Design review of the part built by this model. Coordinates are the model's own, in mm. Face numbers are marked on the shaded views. A direction names the side the tool comes from. Coordinates: 2 decimals unless noted, no trailing zeros. Loops run counter-clockwise (first coordinate to the right, second up) from the corner with the lowest first, then second, coordinate; pieces in that order, holes last. Notation, with made-up numbers: (-17, -22.75) -> (-13, -22.75) arc R18 ccw to (-13, -1.75) -> close; hole circle Ø11 at (55.5, 44). An arc over 180 degrees is marked (long way). Use one line per item in the form item = value. Start each with the question number.
1. Consider section D-D (y = 22.75). State the section outline as (x, z) points (3 decimals).
2. For pin 1 (5.5 mm diameter, centred on y = 18.5, z = 6.5, fed in from -X); pin 2 (1 mm diameter, centred on y = 11.5, z = 15, fed in from +X); pin 3 (5 mm diameter, centred on y = 11, z = 5.5, fed in from +X), all flat-tipped, find the tip position at first contact; note any pin that passes through.
3. Machinability: for the marked faces 1, 2 and 3, which of the approach directions +Z, -Z, +X, -X, +Y, -Y give a long, thin tool a straight path to every point of the face, cutting with its end or side? Answer none if there is none.
4. Wall thickness on line 1 (X direction, y = 2.8, z = 12.5); line 2 (X direction, y = 18.25, z = 17); line 3 (Y direction, x = 16.5, z = 5): over which ranges is each line inside the solid? List them lowest first. Write a range as from..to.
5. The part is to be moulded in two halves that separate along X. For the marked faces 4, 5, 6 and 7, say which applies: released by +X, released by -X, zero draft, split by the parting line, or undercut.
6. Consider section A-A (z = 3). State the section outline as (x, y) points, then the cut area to 3 significant figures.
7. Consider section C-C (z = 14.25). State the section outline as (x, y) points, then the cut area to 3 significant figures.
8. Consider section B-B (x = 7.5). State the section outline as (y, z) points, then the cut area to 3 significant figures.
from build123d import *

# Parameters (mm, degrees)
BASE_PROFILE_SKETCH_W      = 40
BASE_PROFILE_SKETCH_H      = 6
BASE_BODY_DEPTH            = 25
UPRIGHT_BLOCK_SKETCH_W     = 6
UPRIGHT_BLOCK_SKETCH_H     = 15
UPRIGHT_BLOCK_DEPTH        = 25
SLOTTED_CLEVIS_PLATE_DEPTH = 6
LUG_1_DEPTH                = 5
LUG_1_PIN_HOLE_SKETCH_R    = 1.25
LUG_1_PIN_HOLE_DEPTH       = 5
LUG_START                  = -5
LUG_2_DEPTH                = 5
LUG_2_PIN_HOLE_SKETCH_R    = 1.25
LUG_2_PIN_HOLE_DEPTH       = 5
MOUNTING_HOLES_SKETCH_R    = 3
MOUNTING_HOLES_2X_6_DEPTH  = 6


with BuildPart() as part:
    # Base Profile Sketch → Base Body (new body)
    with BuildSketch(Plane.XY):
        with Locations((20, 3)):
            Rectangle(BASE_PROFILE_SKETCH_W, BASE_PROFILE_SKETCH_H)
    extrude(amount=BASE_BODY_DEPTH)

    # Upright Block Sketch → Upright Block (add)
    with BuildSketch(Plane.XY.offset(25)):
        with Locations((43, 7.5)):
            Rectangle(UPRIGHT_BLOCK_SKETCH_W, UPRIGHT_BLOCK_SKETCH_H)
    extrude(amount=-UPRIGHT_BLOCK_DEPTH)

    # Clevis Slot Profile Sketch → Slotted Clevis Plate (add)
    with BuildSketch(Plane.ZY.offset(-40)):
        with BuildLine():
            ThreePointArc((16, 18.5), (14.974873734, 16.025126266), (12.5, 15))
            Line((12.5, 15), (25, 15))
            Line((25, 15), (20, 25))
            Line((20, 25), (16, 25))
            Line((16, 25), (16, 18.5))
        make_face()
        with BuildLine():
            ThreePointArc((12.5, 15), (10.025126266, 16.025126266), (9, 18.5))
            Line((9, 18.5), (9, 25))
            Line((9, 25), (5, 25))
            Line((5, 25), (0, 15))
            Line((0, 15), (12.5, 15))
        make_face()
    extrude(amount=-SLOTTED_CLEVIS_PLATE_DEPTH)

    # Lug 1 Sketch → Lug 1 (add)
    with BuildSketch(Plane.XY.offset(25)):
        with BuildLine():
            Line((46, 0), (53, 0))
            ThreePointArc((53, 0), (55.757828687, 1.81916092), (55.171034593, 5.070412712))
            Line((55.171034593, 5.070412712), (46, 15))
            Line((46, 15), (46, 0))
        make_face()
    extrude(amount=-LUG_1_DEPTH)

    # Lug 1 Pin Hole Sketch → Lug 1 Pin Hole (cut)
    with BuildSketch(Plane.XY.offset(25)):
        with Locations((53, 3)):
            Circle(LUG_1_PIN_HOLE_SKETCH_R)
    extrude(amount=-LUG_1_PIN_HOLE_DEPTH, mode=Mode.SUBTRACT)

    # Lug 2 Sketch → Lug 2 (add)
    with BuildSketch(Plane(origin=(0, 0, 0), x_dir=(-1, 0, 0), z_dir=(0, 0, -1)).offset(LUG_START)):
        with BuildLine():
            Line((-46, 0), (-53, 0))
            ThreePointArc((-53, 0), (-55.757828687, 1.81916092), (-55.171034593, 5.070412712))
            Line((-55.171034593, 5.070412712), (-46, 15))
            Line((-46, 15), (-46, 0))
        make_face()
    extrude(amount=LUG_2_DEPTH)

    # Lug 2 Pin Hole Sketch → Lug 2 Pin Hole (cut)
    with BuildSketch(Plane(origin=(0, 0, 0), x_dir=(-1, 0, 0), z_dir=(0, 0, -1)).offset(LUG_START)):
        with Locations(Location((-53, 3, 0), (0, 0, 180))):
            Circle(LUG_2_PIN_HOLE_SKETCH_R)
    extrude(amount=LUG_2_PIN_HOLE_DEPTH, mode=Mode.SUBTRACT)

    # Mounting Holes Sketch → Mounting Holes 2xØ6 (cut)
    with BuildSketch(Plane(origin=(0, 6, 0), x_dir=(1, 0, 0), z_dir=(0, 1, 0))):
        with Locations(Location((7.5, -12.5, 0), (0, 0, 270))):
            Circle(MOUNTING_HOLES_SKETCH_R)
        with Locations(Location((25, -12.5, 0), (0, 0, 270))):
            Circle(MOUNTING_HOLES_SKETCH_R)
    extrude(amount=-MOUNTING_HOLES_2X_6_DEPTH, mode=Mode.SUBTRACT)


solid = part.part
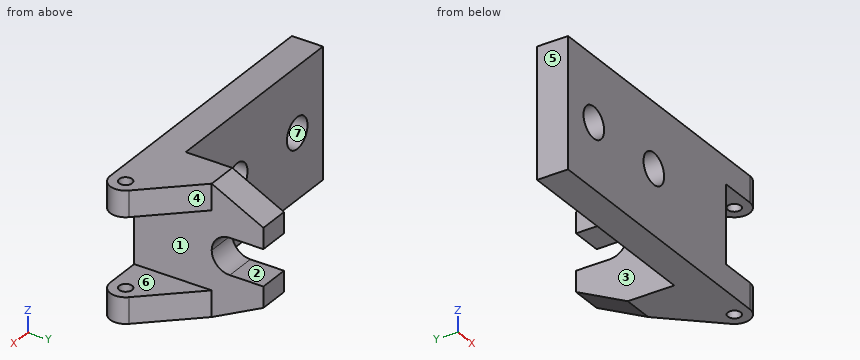
Geometry check:
q1.outline = (40, 3.875) -> (46, 3.875) -> (46, 9) -> (40, 9) -> close; (40, 16) -> (46, 16) -> (46, 21.125) -> (40, 21.125) -> close
q2.pin_1 = 40
q2.pin_2 = 46
q2.pin_3 = 51.96
q3.face_1 = +X, +Y
q3.face_2 = +X, -X, +Y
q3.face_3 = +Z, -Z, -X, +Y
q4.line_1 = 0..4.5, 10.5..22, 28..46
q4.line_2 = 40..46
q4.line_3 = 0..6
q5.face_4 = released by +X
q5.face_5 = released by -X
q5.face_6 = zero draft
q5.face_7 = undercut
q6.outline = (0, 0) -> (53, 0) arc R3 ccw to (55.17, 5.07) -> (46, 15) -> (46, 21) -> (40, 21) -> (40, 6) -> (0, 6) -> close; hole circle Ø2.5 at (53, 3)
q6.area = 455 mm²
q7.outline = (0, 0) -> (5.06, 0) -> (5.06, 6) -> (0, 6) -> close; (9.94, 0) -> (22.56, 0) -> (22.56, 6) -> (9.94, 6) -> close; (27.44, 0) -> (46, 0) -> (46, 15.47) -> (40, 15.47) -> (40, 6) -> (27.44, 6) -> close
q7.area = 274 mm²
q8.outline = (0, 0) -> (6, 0) -> (6, 9.5) -> (0, 9.5) -> close; (0, 15.5) -> (6, 15.5) -> (6, 25) -> (0, 25) -> close
q8.area = 114 mm²
